The model under review builds one solid part; all positions refer to its coordinate system, in mm. Give positions to 0.01 mm unless a question says otherwise; leave off trailing zeros. Loops run counter-clockwise (first coordinate to the right, second up) from the corner with the lowest first, then second, coordinate; pieces in that order, holes last. Notation, with made-up numbers: M 68,71 L 121,71 A21 ccw 121,84 Z; hole C 70,-36 d2. An arc over 180 degrees is marked long. Put each result on its own line as item: value. Start each with the question number.
from build123d import *

# Parameters (mm, degrees)
BOSS_EXTRUDE1_DEPTH = 8


with BuildPart() as part:
    # Sketch1 → Boss-Extrude1 (new body)
    with BuildSketch(Plane.XY):
        Polygon((10, 66), (110, 10), (110, 0), (0, 0), (0, 66), align=None)
    extrude(amount=BOSS_EXTRUDE1_DEPTH)


solid = part.part
(1) To check wall thickness, follow L1, parallel to X at y = 13, z = 5.5; L2, parallel to Y at x = 44, z = 5.5; L3, parallel to X at y = 61.5, z = 1.5. State the ranges of each line that lie inside material, in increasing order. Write a range as [from, to].
(2) We need section C-C, the plane y = 48.5. Write out the cut boundary in (x, z).
(3) We need section B-B, the plane x = 40.5. Write out the cut boundary in (y, z).
(4) Insertion check: pin 1 (1.5 mm diameter, centred on y = 19, z = 6.5, fed in from +X). The pin has a flat end and moves straight along its axis. Give the tip position at first contact, or say it passes through.
(5) We need section A-A, the plane z = 3.75. Write out the cut boundary in (x, y).
Check sheet entries:
1. L1: x = [0, 104.64]
1. L2: y = [0, 46.96]
1. L3: x = [0, 18.04]
2. outline: M 0,0 L 41.25,0 L 41.25,8 L 0,8 Z
3. outline: M 0,0 L 48.92,0 L 48.92,8 L 0,8 Z
4. pin 1: stops at x = 95.27
5. outline: M 0,0 L 110,0 L 110,10 L 10,66 L 0,66 Z
